```python
from build123d import *

# Parameters (mm, degrees)
SKETCH_1_W          = 667
SKETCH_1_H          = 791
EXTRUDE_1_DEPTH     = 50
SKETCH_6_W          = 516
SKETCH_6_H          = 164
CUT_EXTRUDE_1_DEPTH = 520.752344872
SKETCH_4_W          = 751
SKETCH_4_H          = 50
EXTRUDE_2_DEPTH     = 92
SKETCH_5_W          = 751
SKETCH_5_H          = 50
EXTRUDE_3_DEPTH     = 92
SHELL_2_T           = -2
FILLET_1_R          = 1
FILLET_2_R          = 3
FILLET_3_R          = 5
FILLET_4_R          = 28
FILLET_5_R          = 30
SKETCH_7_W          = 447
SKETCH_7_H          = 12
CUT_EXTRUDE_2_DEPTH = 2
SKETCH_8_W          = 447
SKETCH_8_H          = 12
CUT_EXTRUDE_3_DEPTH = 2
SKETCH_9_W          = 547
SKETCH_9_H          = 12
CUT_EXTRUDE_4_DEPTH = 2
SKETCH_10_W         = 450
SKETCH_10_H         = 12
CUT_EXTRUDE_5_DEPTH = 50


with BuildPart() as part:
    # 草图1 → 凸台-拉伸1 (new body)
    with BuildSketch(Plane(origin=(0, 0, 0), x_dir=(1, 0, 0), z_dir=(0, 1, 0))):
        Rectangle(SKETCH_1_W, SKETCH_1_H)
    extrude(amount=EXTRUDE_1_DEPTH)

    # 草图6 → 切除-拉伸1 (cut, through all)
    with BuildSketch(Plane(origin=(0, 50, 0), x_dir=(1, 0, 0), z_dir=(0, 1, 0))):
        with Locations((0, -313.5)):
            Rectangle(SKETCH_6_W, SKETCH_6_H)
    extrude(amount=-CUT_EXTRUDE_1_DEPTH, mode=Mode.SUBTRACT)

    # 草图4 → 凸台-拉伸2 (add)
    with BuildSketch(Plane(origin=(333.5, 0, 0), x_dir=(0, 0, -1), z_dir=(1, 0, 0))):
        with Locations((20, 25)):
            Rectangle(SKETCH_4_W, SKETCH_4_H)
    extrude(amount=EXTRUDE_2_DEPTH)

    # 草图5 → 凸台-拉伸3 (add)
    with BuildSketch(Plane.ZY.offset(333.5)):
        with Locations((-20, 25)):
            Rectangle(SKETCH_5_W, SKETCH_5_H)
    extrude(amount=EXTRUDE_3_DEPTH)

    # 抽壳2
    shell_2_openings = [part.faces().sort_by_distance(p)[0] for p in [
        (0, 50, -50.405146974),
        (0, 0, -50.405146974),
    ]]
    offset(amount=SHELL_2_T, openings=shell_2_openings, kind=Kind.INTERSECTION)

    # 圆角1
    fillet_1_edges = [part.edges().sort_by_distance(p)[0] for p in [
        (331.5, 25, 393.5),
        (-260, 25, 393.5),
        (-331.5, 25, 393.5),
        (260, 25, 393.5),
        (423.5, 25, 353.5),
        (423.5, 25, -393.5),
        (-423.5, 25, -393.5),
        (-423.5, 25, 353.5),
    ]]
    fillet(fillet_1_edges, radius=FILLET_1_R)

    # 圆角2
    fillet_2_edges = [part.edges().sort_by_distance(p)[0] for p in [
        (-333.5, 25, 355.5),
        (333.5, 25, 355.5),
        (425.5, 25, 355.5),
        (425.5, 25, -395.5),
        (-425.5, 25, -395.5),
        (-425.5, 25, 355.5),
        (333.5, 25, 395.5),
        (-333.5, 25, 395.5),
        (258, 25, 395.5),
        (-258, 25, 395.5),
    ]]
    fillet(fillet_2_edges, radius=FILLET_2_R)

    # 圆角3
    fillet_3_edges = [part.edges().sort_by_distance(p)[0] for p in [
        (331.5, 25, 353.5),
        (-331.5, 25, 353.5),
    ]]
    fillet(fillet_3_edges, radius=FILLET_3_R)

    # 圆角4
    fillet_4_edges = [part.edges().sort_by_distance(p)[0] for p in [
        (-258, 25, 231.5),
        (258, 25, 231.5),
    ]]
    fillet(fillet_4_edges, radius=FILLET_4_R)

    # 圆角5
    fillet_5_edges = [part.edges().sort_by_distance(p)[0] for p in [
        (-260, 25, 229.5),
        (260, 25, 229.5),
    ]]
    fillet(fillet_5_edges, radius=FILLET_5_R)

    # 草图7 → 切除-拉伸2 (cut)
    with BuildSketch(Plane(origin=(425.5, 0, 0), x_dir=(0, 0, -1), z_dir=(1, 0, 0))):
        with Locations((20, 6)):
            Rectangle(SKETCH_7_W, SKETCH_7_H)
    extrude(amount=-CUT_EXTRUDE_2_DEPTH, mode=Mode.SUBTRACT)

    # 草图8 → 切除-拉伸3 (cut)
    with BuildSketch(Plane.ZY.offset(425.5)):
        with Locations((-20, 6)):
            Rectangle(SKETCH_8_W, SKETCH_8_H)
    extrude(amount=-CUT_EXTRUDE_3_DEPTH, mode=Mode.SUBTRACT)

    # 草图9 → 切除-拉伸4 (cut)
    with BuildSketch(Plane(origin=(0, 0, -395.5), x_dir=(-1, 0, 0), z_dir=(0, 0, -1))):
        with Locations((0, 6)):
            Rectangle(SKETCH_9_W, SKETCH_9_H)
    extrude(amount=-CUT_EXTRUDE_4_DEPTH, mode=Mode.SUBTRACT)

    # 草图10 → 切除-拉伸5 (cut, symmetric)
    with BuildSketch(Plane.XY.offset(231.5)):
        with Locations((0, 6)):
            Rectangle(SKETCH_10_W, SKETCH_10_H)
    extrude(amount=CUT_EXTRUDE_5_DEPTH, both=True, mode=Mode.SUBTRACT)


solid = part.part
```
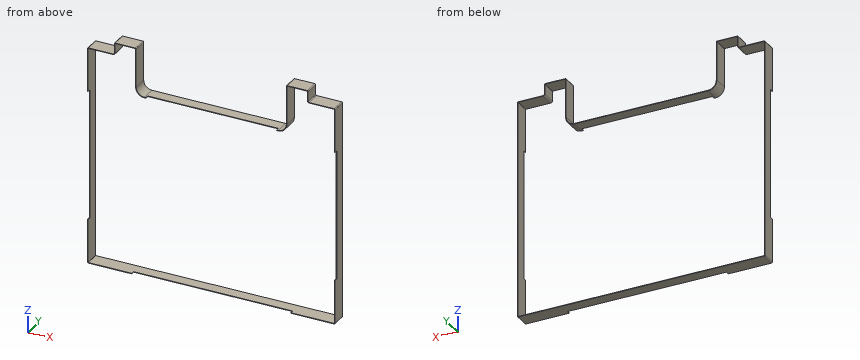
Build history of the part. All positions in model axes, mm. Coordinates: 2 decimals unless noted, no trailing zeros. Write each loop counter-clockwise with the first axis right and the second up, starting at its lowest first coordinate (ties: lowest second). Pieces come first, ordered by that corner, then holes.
1. Drop flat-ended pins along their axis: pin 1 (1.6 mm diameter, centred on x = 14.5, z = 230, fed in from -Y); pin 2 (25 mm diameter, centred on x = 118.5, y = 34.5, fed in from +Z); pin 3 (1 mm diameter, centred on x = -425, y = 9, fed in from -Z). Give the stop position or say it passes through.
Answer block:
pin 1: stops at y = 12
pin 2: stops at z = 231.5
pin 3: stops at z = -394.74
2. Band-saw the part on A-A, the plane z = -277.5. Give the cut face in (x, y), and give its area (3 significant figures).
Answer block:
outline: (-425.5, 0) - (-423.5, 0) - (-423.5, 50) - (-425.5, 50) - close; (423.5, 0) - (425.5, 0) - (425.5, 50) - (423.5, 50) - close
area: 200 mm2
3. Drill centre lines: probe 1 along X at (y, z) = (36, 266); probe 2 along Z at (x, y) = (307, 35); probe 3 along Z at (x, y) = (360, 33). Where is each one in solid material? Low to high.
Answer block:
probe 1: x = -425.5 to -423.5, -260 to -258, 258 to 260, 423.5 to 425.5
probe 2: z = -395.5 to -393.5, 393.5 to 395.5
probe 3: z = -395.5 to -393.5, 353.5 to 355.5
4. Band-saw the part on B-B, the plane x = -197. Give the cut face in (y, z).
Answer block:
outline: (12, -395.5) - (50, -395.5) - (50, -393.5) - (12, -393.5) - close; (12, 229.5) - (50, 229.5) - (50, 231.5) - (12, 231.5) - close
